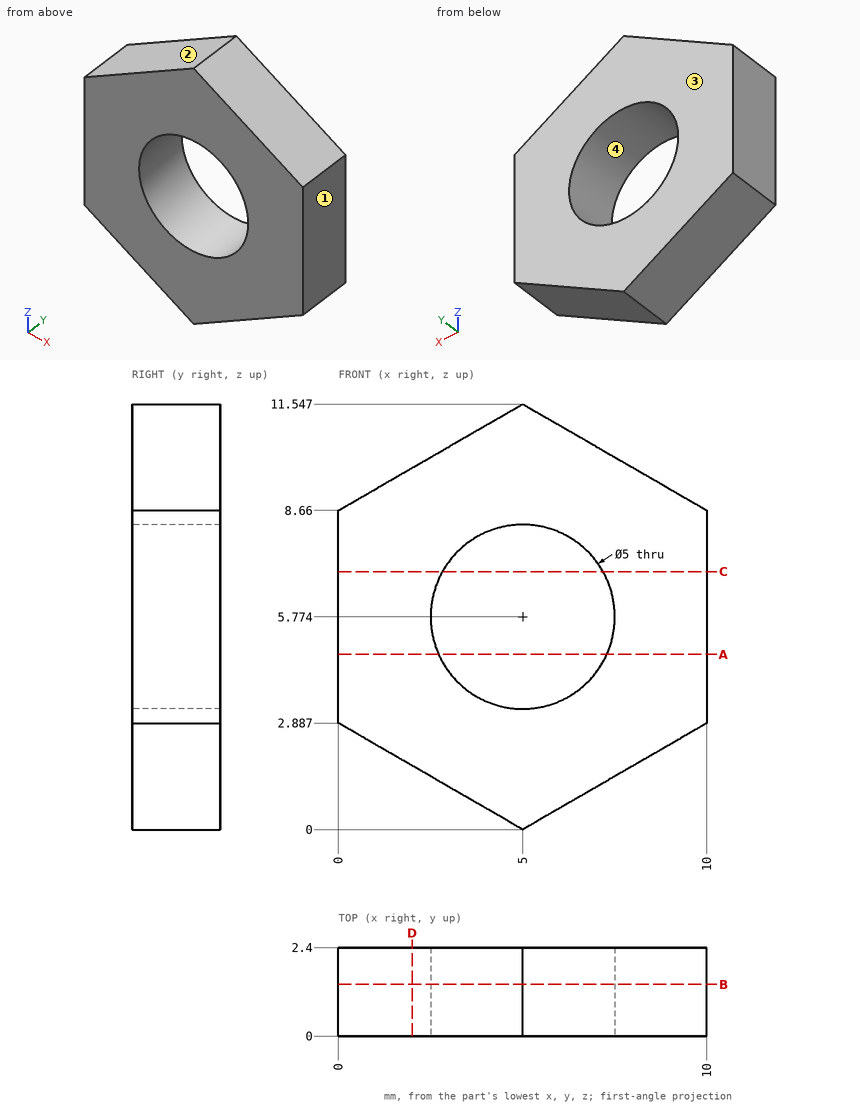
For this review, use the dimensioned drawing (mm, ordinates from the lowest corner) and the shaded views. Coordinates: 2 decimals unless noted, no trailing zeros. Loops run counter-clockwise (first coordinate to the right, second up) from the corner with the lowest first, then second, coordinate; pieces in that order, holes last.
1. Add section B-B, the plane y = 1.4. Give the boundary of the cut face in (x, z).
2. Add section A-A, the plane z = 4.75. Give the boundary of the cut face in (x, y).
3. For line 1 (X direction, y = 1.2, z = 5.5) (1 decimal); line 2 (Z direction, x = 6, y = 1.65) (1 decimal); line 3 (Z direction, x = 5.75, y = 2.15) (1 decimal), list the stretches that pass through material, from the lowest coordinate up.
4. Mouldability with a two-part tool opening along X and no side actions: class the marked faces 1, 2, 3 and 4 as +X half, -X half, draft (parallel to the pull), parting line (faces both ways), or undercut.
5. Add section D-D, the plane x = 2. Give the boundary of the cut face in (y, z) (1 decimal).
6. Add section C-C, the plane z = 7. Give the boundary of the cut face in (x, y).
Result:
1. outline: (0, 2.89) - (5, 0) - (10, 2.89) - (10, 8.66) - (5, 11.55) - (0, 8.66) - close; hole circle Ø5 at (5, 5.77)
2. outline: (0, 0) - (2.72, 0) - (2.72, 2.4) - (0, 2.4) - close; (7.28, 0) - (10, 0) - (10, 2.4) - (7.28, 2.4) - close
3. line 1: x = 0 to 2.5, 7.5 to 10
3. line 2: z = 0.6 to 3.5, 8.1 to 11
3. line 3: z = 0.4 to 3.4, 8.2 to 11.1
4. face 1: +X half
4. face 2: -X half
4. face 3: draft
4. face 4: undercut
5. outline: (0, 1.7) - (2.4, 1.7) - (2.4, 9.8) - (0, 9.8) - close
6. outline: (0, 0) - (2.82, 0) - (2.82, 2.4) - (0, 2.4) - close; (7.18, 0) - (10, 0) - (10, 2.4) - (7.18, 2.4) - close
